Could you check a few things on this drawing? It's one solid part, dimensions in mm from its lowest x, y, z. A direction names the side the tool comes from. Coordinates: 2 decimals unless noted, no trailing zeros. Order: outer loops, then holes, each group sorted by start corner. A loop starts at its lowest first (then second) coordinate and runs counter-clockwise, first axis right, second up. Notation, with made-up numbers: (66.5, 31) -> (124.5, 31) arc R24 cw to (124.5, 61) -> close; hole circle Ø7 at (55.25, -32). An arc over 180 degrees is marked (long way). Use a Markdown table: item, result. Add a question column.
1. Suppose I cut it at C-C, the plane x = 40. List the corners of the cut face in (y, z) for me, then the cut area to 3 significant figures.
2. Suppose I cut it at D-D, the plane z = 5. List the corners of the cut face in (x, y) for me, then the cut area to 3 significant figures.
3. For pin 1 Ø10 at (x, z) = (50, 29) entering from -Y; pin 2 Ø3.5 at (x, y) = (40, 10) entering from +Z; pin 3 Ø10 at (x, y) = (75, 13.5) entering from +Z; pin 4 Ø10 at (y, z) = (22, 46) entering from -X, each with a flat end and sliding along its axis, tell me the tip position at first contact or that it passes through.
4. If I drill on line 1 along X through (y, z) = (24.75, 32); line 2 along X through (y, z) = (10, 2.75); line 3 along Z through (x, y) = (85, 25.75), over which ranges is the centre line in solid material (lowest first)? Write a range as from..to.
5. Suppose I cut it at A-A, the plane y = 10. List the corners of the cut face in (x, z) for me, then the cut area to 3 significant figures.
6. For the marked faces 1 and 2, which set-ups out of +Z, -Z, +X, -X, +Y, -Y let a thin tool reach every point of the face, with its end or its side?
7. Suppose I cut it at B-B, the plane z = 32. List the corners of the cut face in (x, y) for me, then the cut area to 3 significant figures.
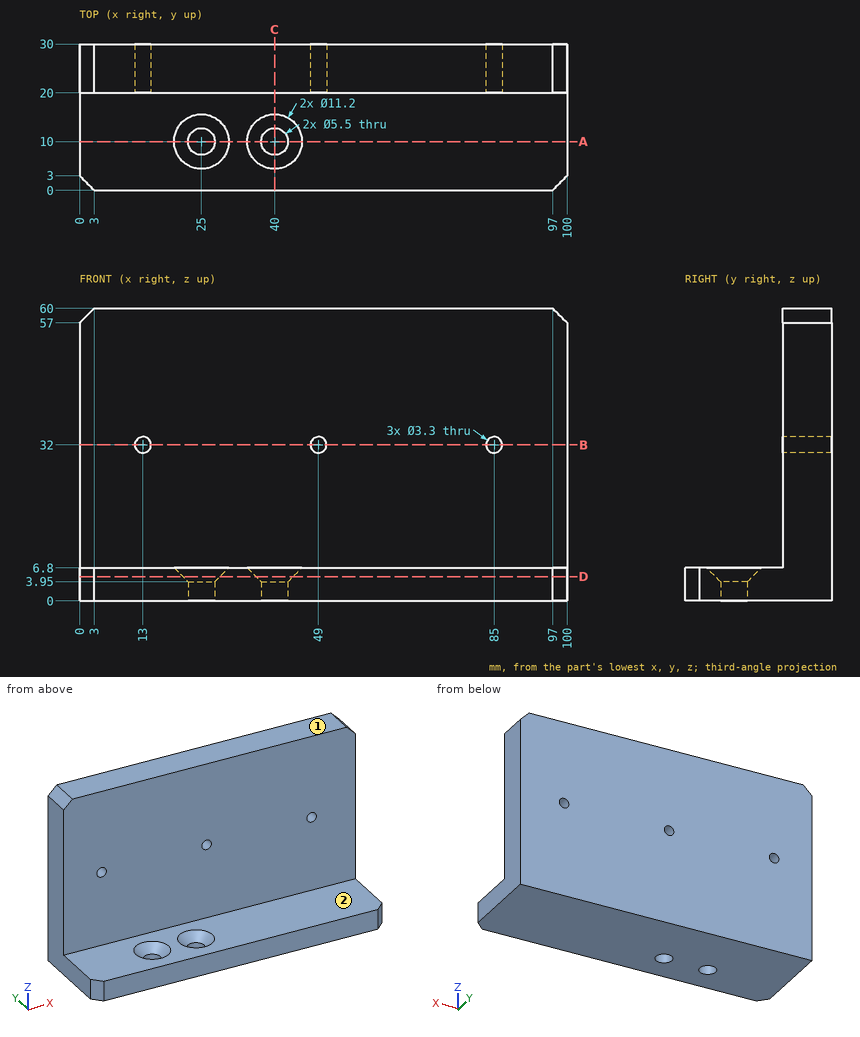
Worked out:
| question | item | result |
|---|---|---|
| 1 | outline | (0, 0) -> (7.25, 0) -> (7.25, 3.95) -> (4.4, 6.8) -> (0, 6.8) -> close; (12.75, 0) -> (30, 0) -> (30, 60) -> (20, 60) -> (20, 6.8) -> (15.6, 6.8) -> (12.75, 3.95) -> close |
| 1 | area | 690 mm² |
| 2 | outline | (0, 3) -> (3, 0) -> (97, 0) -> (100, 3) -> (100, 30) -> (0, 30) -> close; hole circle Ø7.6 at (25, 10); hole circle Ø7.6 at (40, 10) |
| 2 | area | 2,900 mm² |
| 3 | pin 1 | stops at y = 20 |
| 3 | pin 2 | passes through |
| 3 | pin 3 | stops at z = 6.8 |
| 3 | pin 4 | stops at x = 0 |
| 4 | line 1 | x = 0..11.35, 14.65..47.35, 50.65..83.35, 86.65..100 |
| 4 | line 2 | x = 0..22.25, 27.75..37.25, 42.75..100 |
| 4 | line 3 | z = 0..30.35, 33.65..60 |
| 5 | outline | (0, 0) -> (22.25, 0) -> (22.25, 3.95) -> (19.4, 6.8) -> (0, 6.8) -> close; (27.75, 0) -> (37.25, 0) -> (37.25, 3.95) -> (34.4, 6.8) -> (30.6, 6.8) -> (27.75, 3.95) -> close; (42.75, 0) -> (100, 0) -> (100, 6.8) -> (45.6, 6.8) -> (42.75, 3.95) -> close |
| 5 | area | 589 mm² |
| 6 | face 1 | +Z, +X, -X, +Y, -Y |
| 6 | face 2 | +Z, +X, -X, -Y |
| 7 | outline | (0, 20) -> (11.35, 20) -> (11.35, 30) -> (0, 30) -> close; (14.65, 20) -> (47.35, 20) -> (47.35, 30) -> (14.65, 30) -> close; (50.65, 20) -> (83.35, 20) -> (83.35, 30) -> (50.65, 30) -> close; (86.65, 20) -> (100, 20) -> (100, 30) -> (86.65, 30) -> close |
| 7 | area | 901 mm² |
